from build123d import *

# Parameters (mm, degrees)
EXTRUDE_1_DEPTH     = 30
SKETCH_3_R          = 103
SKETCH_3_R_2        = 93
EXTRUDE_2_DEPTH     = 85
CHAMFER_1_SIZE      = 2
CHAMFER_1_SIZE2     = 2.444922552
CHAMFER_2_SIZE      = 2
SKETCH_5_W          = 50
SKETCH_5_H          = 65
SKETCH_5_W_2        = 51
SKETCH_5_H_2        = 60
CUT_EXTRUDE_1_DEPTH = 145
CUT_EXTRUDE_2_REACH = 738.023
SKETCH_6_R          = 6.5
SKETCH_7_W          = 8
SKETCH_7_H          = 290.552201754
SKETCH_7_H_2        = 289.758517494
CUT_EXTRUDE_3_DEPTH = 30


with BuildPart() as part:
    # 草图2 → 凸台-拉伸1 (new body)
    with BuildSketch(Plane.XY):
        with BuildLine():
            Line((-107.5, 21.352049082), (-107.5, -186.717950918))
            ThreePointArc((-107.5, -186.717950918), (0, -232.105571153), (107.5, -186.717950918))
            Line((107.5, -186.717950918), (107.5, 21.352049082))
            ThreePointArc((107.5, 21.352049082), (0, 109.6), (-107.5, 21.352049082))
        make_face()
    extrude(amount=EXTRUDE_1_DEPTH)

    # 草图3 → 凸台-拉伸2 (add)
    with BuildSketch(Plane(origin=(0, 0, 0), x_dir=(-1, 0, 0), z_dir=(0, 0, -1))):
        with Locations(Location((0, -82.682950918, 0), (0, 0, 180))):
            Circle(SKETCH_3_R)
        with Locations((0, -82.682950918)):
            Circle(SKETCH_3_R_2, mode=Mode.SUBTRACT)
    extrude(amount=EXTRUDE_2_DEPTH)

    # 草图4 → 旋转1 (revolve)
    with BuildSketch(Plane.ZX.offset(-82.682950918)):
        Polygon((-95, -93), (-95, -122), (-213, -122), (-213, -110), (-303, -110), (-303, -95), (-438, -95), (-438, -124.5), (-477, -124.5), (-477, -90), (-485, -90), (-485, -77.5), (-655, -77.5), (-655, -89.5), (-497, -89.5), (-489, -136.5), (-426, -136.5), (-426, -107), (-343, -107), (-315, -122), (-225, -122), (-225, -134), (-83, -134), (-83, -93), align=None)
    revolve(axis=Axis((0, -82.682950918, -1172.450178842), (0, 0, 1)))

    # 倒角1
    chamfer_1_edges = [part.edges().sort_by_distance(p)[0] for p in [
        (136.5, -82.682950918, -489),
    ]]
    chamfer_1_side = [part.faces().sort_by_distance(p)[0] for p in [
        (136.5, -82.682950918, -457.5),
    ]]
    chamfer(chamfer_1_edges, length=CHAMFER_1_SIZE, length2=CHAMFER_1_SIZE2, reference=chamfer_1_side[0])

    # 倒角2
    chamfer_2_edges = [part.edges().sort_by_distance(p)[0] for p in [
        (134, -82.682950918, -83),
        (134, -82.682950918, -225),
        (136.5, -82.682950918, -426),
    ]]
    chamfer(chamfer_2_edges, length=CHAMFER_2_SIZE)

    # 草图5 → 切除-拉伸1 (cut)
    with BuildSketch(Plane.ZX.offset(-82.682950918)):
        with Locations((-250, 0)):
            Rectangle(SKETCH_5_W, SKETCH_5_H)
        with Locations((-400.5, 0)):
            Rectangle(SKETCH_5_W_2, SKETCH_5_H_2)
    extrude(amount=CUT_EXTRUDE_1_DEPTH, mode=Mode.SUBTRACT)

    # 草图6 → 切除-拉伸2 (cut, up to next)
    with BuildSketch(Plane.XY.offset(30), mode=Mode.PRIVATE) as cut_extrude_2_sk1:
        with Locations((0, 42.317049082)):
            Circle(SKETCH_6_R)
    cut_extrude_2_tool1 = extrude(cut_extrude_2_sk1.sketch, amount=-CUT_EXTRUDE_2_REACH, mode=Mode.PRIVATE) & part.part
    # 草图6 → 切除-拉伸2 (cut, up to next)
    with BuildSketch(Plane.XY.offset(30), mode=Mode.PRIVATE) as cut_extrude_2_sk2:
        with Locations((0, -207.682950918)):
            Circle(SKETCH_6_R)
    cut_extrude_2_tool2 = extrude(cut_extrude_2_sk2.sketch, amount=-CUT_EXTRUDE_2_REACH, mode=Mode.PRIVATE) & part.part
    # 草图6 → 切除-拉伸2 (cut, up to next)
    with BuildSketch(Plane.XY.offset(30), mode=Mode.PRIVATE) as cut_extrude_2_sk3:
        with Locations((-76.315136113, -181.682950918)):
            Circle(SKETCH_6_R)
    cut_extrude_2_tool3 = extrude(cut_extrude_2_sk3.sketch, amount=-CUT_EXTRUDE_2_REACH, mode=Mode.PRIVATE) & part.part
    # 草图6 → 切除-拉伸2 (cut, up to next)
    with BuildSketch(Plane.XY.offset(30), mode=Mode.PRIVATE) as cut_extrude_2_sk4:
        with Locations((76.315136113, -181.682950918)):
            Circle(SKETCH_6_R)
    cut_extrude_2_tool4 = extrude(cut_extrude_2_sk4.sketch, amount=-CUT_EXTRUDE_2_REACH, mode=Mode.PRIVATE) & part.part
    add(cut_extrude_2_tool1.solids().sort_by_distance((0, 42.317049, 30))[0], mode=Mode.SUBTRACT)
    add(cut_extrude_2_tool2.solids().sort_by_distance((0, -207.682951, 30))[0], mode=Mode.SUBTRACT)
    add(cut_extrude_2_tool3.solids().sort_by_distance((-76.315136, -181.682951, 30))[0], mode=Mode.SUBTRACT)
    add(cut_extrude_2_tool4.solids().sort_by_distance((76.315136, -181.682951, 30))[0], mode=Mode.SUBTRACT)

    # 草图7 → 切除-拉伸3 (cut)
    with BuildSketch(Plane.XY.offset(30)):
        with Locations((-103.5, -82.682950918)):
            Rectangle(SKETCH_7_W, SKETCH_7_H)
        with Locations((103.5, -82.682950918)):
            Rectangle(SKETCH_7_W, SKETCH_7_H_2)
    extrude(amount=-CUT_EXTRUDE_3_DEPTH, mode=Mode.SUBTRACT)


solid = part.part
Geometry: final body of the model. Coordinates: model frame, mm. A direction names the side the tool comes from. Give positions to 0.01 mm unless a question says otherwise; leave off trailing zeros. Write each loop counter-clockwise with the first axis right and the second up, starting at its lowest first coordinate (ties: lowest second). Pieces come first, ordered by that corner, then holes. Notation, with made-up numbers: (-14.75, 46) -> (27.25, 46) arc R31 ccw to (27.25, 83) -> close; hole circle Ø7 at (-13.75, 65). An arc over 180 degrees is marked (long way). Answer in a Markdown table with one row per item.
(1) Section query B-B on x = -20. State how many separate pieces and enclosed holes the cut face has, then the cut area to 3 significant figures.
Answers below:
| item | result |
|---|---|
| separate pieces | 3 |
| enclosed holes | 0 |
| area | 28,400 mm^2 |
(2) Section query A-A on z = -293.5. Return loops of the section in (x, y).
Answers below:
| item | result |
|---|---|
| outline | circle Ø244 at (0, -82.68); hole circle Ø220 at (0, -82.68) |
(3) Section query C-C on y = 73.5. Return loops of the section in (x, z), then the cut area to 3 significant figures.
Answers below:
| item | result |
|---|---|
| outline | (-81.3, 0) -> (81.3, 0) -> (81.3, 30) -> (-81.3, 30) -> close |
| area | 4,880 mm^2 |
(4) Pin query (flat end, axial travel): pin 1 (1 mm diameter, centred on x = 101.5, y = -90.5, fed in from +Z); pin 2 (6 mm diameter, centred on x = -70, z = -540, fed in from +Y); pin 3 (21 mm diameter, centred on x = 0, y = -207.68, fed in from +Z); pin 4 (3 mm diameter, centred on y = -161, z = -84, fed in from +X). Return the tip coordinate at first contact, or that it passes through.
Answers below:
| item | result |
|---|---|
| pin 1 | z = 0 |
| pin 2 | y = -23.34 |
| pin 3 | z = 30 |
| pin 4 | x = 109.53 |
(5) Ray query, line 1 along Y through (x, z) = (0, -482); line 2 along Z through (x, y) = (17.5, 16.5); line 3 along Z through (x, y) = (91, -126). Return the intervals inside material, ascending. Write a range as [from, to].
Answers below:
| item | result |
|---|---|
| line 1 | [-219.18, -172.68], [7.32, 53.82] |
| line 2 | [-495.09, -477], [-438, -426], [-375, -303], [-95, 30] |
| line 3 | [-495.08, -477], [-438, -303], [-95, 30] |
(6) Set-up query: faces 4 (the conical face through (-58.027, -173.697, -341.248)), 5 (the cylindrical face through (-77.16, -175.24, 15.21)), 6 (the flat face through (-27, -156, -655)). Return all of +Z, -Z, +X, -X, +Y, -Y with unobstructed straight access to the full face (end or side cutting, diameter ignored); none if empty.
Answers below:
| item | result |
|---|---|
| face 4 | none |
| face 5 | +Z |
| face 6 | -Z, +X, -X, +Y, -Y |
(7) Draft query along X for faces 1 (the flat face through (-78, -15, -83)), 2 (the cylindrical face through (-127.812, -122.933, -153.034)), 3 (the flat face through (-28, 7, -95)). Return one class per face: +X half, -X half, draft (parallel to the pull), parting line (faces both ways), or undercut.
Answers below:
| item | result |
|---|---|
| face 1 | draft |
| face 2 | parting line |
| face 3 | undercut |
(8) Section query D-D on z = -554.5. Return loops of the section in (x, y), then the cut area to 3 significant figures.
Answers below:
| item | result |
|---|---|
| outline | circle Ø179 at (0, -82.68); hole circle Ø155 at (0, -82.68) |
| area | 6,300 mm^2 |
